Input: part model. Units: mm. Frame: model coordinates. Round coordinates to 2 decimals unless told otherwise and drop trailing zeros. Loops run counter-clockwise (first coordinate to the right, second up) from the corner with the lowest first, then second, coordinate; pieces in that order, holes last. Notation, with made-up numbers: (75.5, 7.5) - (108.5, 7.5) arc R22 cw to (108.5, 23.5) - close; hole circle Ø10 at (-21.5, -20.75). An arc over 180 degrees is marked (long way). Use CSV: the item, a comma, the result in double quotes. Start each with the question number.
1. Cut plane B-B (z = 0). Return loops of the section in (x, y).
2. Cut plane A-A (x = 0). Return loops of the section in (y, z).
3. Cut plane D-D (z = -78.5). Return loops of the section in (x, y), and give its area (3 significant figures).
4. Pull-direction query (Z, two-part tool) for faces 1 (the cylindrical face through (-21, 3, -28)), 2 (the cylindrical face through (30.04, 2.71, 95.38)), 3 (the flat face through (-43, 0, -1)); classes: +Z half, -Z half, draft (parallel to the pull), parting line (faces both ways), or undercut.
5. Material intervals for probe 1 along X at (y, z) = (4.8, 0); probe 2 along X at (y, z) = (2.65, 0); probe 3 along X at (y, z) = (0.2, 0), sorted ascending. Write a range as from..to.
6. Cut plane C-C (y = 3.15). Return loops of the section in (x, z).
```python
from build123d import *

# Parameters (mm, degrees)
SKETCH1_R           = 42.5
SKETCH1_R_2         = 35
BOSS_EXTRUDE1_DEPTH = 5.5
CHAMFER1_SIZE       = 1
BOSS_EXTRUDE2_START = -5.5
SKETCH2_R           = 100
SKETCH2_R_2         = 42.5
BOSS_EXTRUDE2_DEPTH = 5.5


with BuildPart() as part:
    # Sketch1 → Boss-Extrude1 (new body)
    with BuildSketch(Plane(origin=(0, 0, 0), x_dir=(1, 0, 0), z_dir=(0, 1, 0))):
        with Locations(Location((0, 0, 0), (0, 0, 270))):
            Circle(SKETCH1_R)
        with Locations(Location((0, 0, 0), (0, 0, 270))):
            Circle(SKETCH1_R_2, mode=Mode.SUBTRACT)
    extrude(amount=BOSS_EXTRUDE1_DEPTH)

    # Chamfer1
    chamfer1_edges = [part.edges().sort_by_distance(p)[0] for p in [
        (0, 0, -42.5),
        (0, 5.5, -42.5),
    ]]
    chamfer(chamfer1_edges, length=CHAMFER1_SIZE)

    # Sketch2 → Boss-Extrude2 (add)
    with BuildSketch(Plane(origin=(0, 5.5, 0), x_dir=(1, 0, 0), z_dir=(0, 1, 0)).offset(BOSS_EXTRUDE2_START)):
        with Locations(Location((0, 0, 0), (0, 0, 270))):
            Circle(SKETCH2_R)
        with Locations(Location((0, 0, 0), (0, 0, 270))):
            Circle(SKETCH2_R_2, mode=Mode.SUBTRACT)
    extrude(amount=BOSS_EXTRUDE2_DEPTH)


solid = part.part
```
Established:
1,outline,"(-100, 0) - (-42.5, 0) - (-42.5, 1) - (-41.5, 0) - (-35, 0) - (-35, 5.5) - (-41.5, 5.5) - (-42.5, 4.5) - (-42.5, 5.5) - (-100, 5.5) - close; (35, 0) - (41.5, 0) - (42.5, 1) - (42.5, 0) - (100, 0) - (100, 5.5) - (42.5, 5.5) - (42.5, 4.5) - (41.5, 5.5) - (35, 5.5) - close"
2,outline,"(0, -100) - (5.5, -100) - (5.5, -42.5) - (4.5, -42.5) - (5.5, -41.5) - (5.5, -35) - (0, -35) - (0, -41.5) - (1, -42.5) - (0, -42.5) - close; (0, 35) - (5.5, 35) - (5.5, 41.5) - (4.5, 42.5) - (5.5, 42.5) - (5.5, 100) - (0, 100) - (0, 42.5) - (1, 42.5) - (0, 41.5) - close"
3,outline,"(-61.95, 0) - (61.95, 0) - (61.95, 5.5) - (-61.95, 5.5) - close"
3,area,"681 mm2"
4,face 1,"undercut"
4,face 2,"parting line"
4,face 3,"draft"
5,probe 1,"x = -100..-42.5, -42.2..-35, 35..42.2, 42.5..100"
5,probe 2,"x = -100..-35, 35..100"
5,probe 3,"x = -100..-42.5, -41.7..-35, 35..41.7, 42.5..100"
6,outline,"circle Ø200 at (0, 0); hole circle Ø70 at (0, 0)"
